Build history of the part. All positions in model axes, mm. A direction names the side the tool comes from. Round coordinates to 2 decimals unless told otherwise and drop trailing zeros. Order: outer loops, then holes, each group sorted by start corner. A loop starts at its lowest first (then second) coordinate and runs counter-clockwise, first axis right, second up. Notation, with made-up numbers: M -22,88 L 5,88 A28 cw 5,107 Z; hole C 75,85.25 d7. An arc over 180 degrees is marked long. Use CSV: the item, a comma, the result in double quotes.
from build123d import *

# Parameters (mm, degrees)
SKETCH1_R              = 39.5
BOSS_EXTRUDE1_DEPTH    = 144
SKETCH2_OUTSIDE_W      = 117.452
SKETCH2_OUTSIDE_H      = 117.452
SKETCH2_OUTSIDE_R      = 22.5
CUT_EXTRUDE1_DEPTH     = 70
SKETCH4_OUTSIDE_W      = 117.452
SKETCH4_OUTSIDE_H      = 117.452
SKETCH4_OUTSIDE_R      = 32.5
CUT_EXTRUDE3_DEPTH     = 45
SKETCH6_OUTSIDE_W      = 117.452
SKETCH6_OUTSIDE_H      = 117.452
SKETCH6_OUTSIDE_R      = 31
CUT_EXTRUDE5_DEPTH     = 10
CHAMFER1_SIZE          = 1
CHAMFER7_SIZE          = 1.5
SKETCH12_R             = 4.25
CUT_EXTRUDE8_DEPTH     = 2
SKETCH15_R             = 63.738357407
CUT_EXTRUDE9_DEPTH     = 70
M42X3_0_TAPPED_HOLE1_D = 39


with BuildPart() as part:
    # Sketch1 → Boss-Extrude1 (new body)
    with BuildSketch(Plane(origin=(0, 0, 0), x_dir=(0, 0, -1), z_dir=(1, 0, 0))):
        Circle(SKETCH1_R)
    extrude(amount=BOSS_EXTRUDE1_DEPTH)

    # Sketch2 outside → Cut-Extrude1 (cut)
    with BuildSketch(Plane(origin=(144, 0, 0), x_dir=(0, 0, -1), z_dir=(1, 0, 0))):
        Rectangle(SKETCH2_OUTSIDE_W, SKETCH2_OUTSIDE_H)
        Circle(SKETCH2_OUTSIDE_R, mode=Mode.SUBTRACT)
    extrude(amount=-CUT_EXTRUDE1_DEPTH, mode=Mode.SUBTRACT)

    # Sketch4 outside → Cut-Extrude3 (cut)
    with BuildSketch(Plane.ZY):
        Rectangle(SKETCH4_OUTSIDE_W, SKETCH4_OUTSIDE_H)
        Circle(SKETCH4_OUTSIDE_R, mode=Mode.SUBTRACT)
    extrude(amount=-CUT_EXTRUDE3_DEPTH, mode=Mode.SUBTRACT)

    # Sketch6 outside → Cut-Extrude5 (cut)
    with BuildSketch(Plane.ZY.offset(-45)):
        Rectangle(SKETCH6_OUTSIDE_W, SKETCH6_OUTSIDE_H)
        Circle(SKETCH6_OUTSIDE_R, mode=Mode.SUBTRACT)
    extrude(amount=CUT_EXTRUDE5_DEPTH, mode=Mode.SUBTRACT)

    # Chamfer1
    chamfer1_edges = [part.edges().sort_by_distance(p)[0] for p in [
        (144, 0, 22.5),
        (0, 0, -32.5),
    ]]
    chamfer(chamfer1_edges, length=CHAMFER1_SIZE)

    # Chamfer7
    chamfer7_edges = [part.edges().sort_by_distance(p)[0] for p in [
        (74, 0, 39.5),
    ]]
    chamfer(chamfer7_edges, length=CHAMFER7_SIZE)

    # Sketch12 → Cut-Extrude8 (cut)
    with BuildSketch(Plane(origin=(0, -39.5, 0), x_dir=(-1, 0, 0), z_dir=(0, -1, 0))):
        with Locations(Location((-60, 0, 0), (0, 0, 90))):
            Circle(SKETCH12_R)
    cut_extrude8 = extrude(amount=-CUT_EXTRUDE8_DEPTH, mode=Mode.SUBTRACT)

    # Sketch14 → M10 Tapped Hole1 (revolve, cut)
    with BuildSketch(Plane(origin=(60, -37.5, 0), x_dir=(0, 0, -1), z_dir=(1, 0, 0))):
        Polygon((0, 0), (0, 12.553657631), (4.25, 10), (4.25, 0), align=None)
    m10_tapped_hole1 = revolve(axis=Axis((60, -43.85, 0), (0, 1, 0)), mode=Mode.SUBTRACT)

    # Mirror1: Cut-Extrude8, M10 Tapped Hole1 across plane
    add(cut_extrude8.mirror(Plane.ZX), mode=Mode.SUBTRACT)
    add(m10_tapped_hole1.mirror(Plane.ZX), mode=Mode.SUBTRACT)

    # Sketch15 → Cut-Extrude9 (cut)
    with BuildSketch(Plane(origin=(144, 0, 0), x_dir=(0, 0, -1), z_dir=(1, 0, 0))):
        Circle(SKETCH15_R)
    extrude(amount=-CUT_EXTRUDE9_DEPTH, mode=Mode.SUBTRACT)

    # M42x3.0 Tapped Hole1 (through all)
    with Locations(Plane(origin=(74, 0, 0), x_dir=(0, 0, -1), z_dir=(1, 0, 0))):
        with Locations((0, 0)):
            Hole(M42X3_0_TAPPED_HOLE1_D / 2)


solid = part.part
(1) Wall check: line 1 (Z direction, x = 66.5, y = 1); line 2 (X direction, y = -38, z = 0); line 3 (Z direction, x = 26.5, y = -1). Give the ranges that are in metal, low to high. Write a range as from..to.
Answer block:
line 1,"z = -39.49..-19.47, 19.47..39.49"
line 2,"x = 45..55.75, 64.25..74"
line 3,"z = -32.48..-19.47, 19.47..32.48"
(2) Two-plate mould, pull along Y, no slides. Class faces 4 (the face through (74, -16, -16)), 5 (the face through (36.482, 19.334, -2.539)), 6 (the face through (59.27, 25.39, 0.1)), 7 (the face through (17.76, 9.76, 31)): released by +Y, released by -Y, zero draft, split by the parting line, or undercut.
Answer block:
face 4,"zero draft"
face 5,"undercut"
face 6,"released by +Y"
face 7,"split by the parting line"
(3) Tool access for faces 1 (the face through (0, 14, -14)), 2 (the face through (40.07, 30.736, -4.036)), 3 (the face through (55.85, 33.58, 0.92)): list every direction of +Z, -Z, +X, -X, +Y, -Y with a clear straight run to the whole face (end or side of a thin tool).
Answer block:
face 1,"+Z, -Z, -X, +Y, -Y"
face 2,"none"
face 3,"+Y"
(4) Drop flat-ended pins along their axis: pin 1 (5 mm diameter, centred on x = 66, z = -26, fed in from +Y); pin 2 (5 mm diameter, centred on x = 60, z = 0, fed in from +Y); pin 3 (6 mm diameter, centred on x = 29, y = -11, fed in from -Z); pin 4 (1 mm diameter, centred on y = 7, z = -17.5, fed in from +X). Give the stop position or say it passes through.
Answer block:
pin 1,"stops at y = 31.75"
pin 2,"stops at y = 26.45"
pin 3,"stops at z = -31.5"
pin 4,"passes through"
(5) Cut at A-A, the plane y = 0. Give the cut face in (x, z).
Answer block:
outline,"M 0,-31.5 L 1,-32.5 L 35,-32.5 L 35,-31 L 45,-31 L 45,-39.5 L 72.5,-39.5 L 74,-38 L 74,-19.5 L 0,-19.5 Z; M 0,19.5 L 74,19.5 L 74,38 L 72.5,39.5 L 45,39.5 L 45,31 L 35,31 L 35,32.5 L 1,32.5 L 0,31.5 Z"
(6) Cut at B-B, the plane x = 53.5. Give the cut face in (y, z).
Answer block:
outline,"C 0,0 d79; hole C 0,0 d39"
